Design review of the part built by this model. Coordinates are the model's own, in mm. A direction names the side the tool comes from. Give positions to 0.01 mm unless a question says otherwise; leave off trailing zeros. Loops run counter-clockwise (first coordinate to the right, second up) from the corner with the lowest first, then second, coordinate; pieces in that order, holes last.
from build123d import *

# Parameters (mm, degrees)
SKETCH_1_R      = 6
EXTRUDE_1_DEPTH = 120
SKETCH_2_R      = 4
EXTRUDE_2_DEPTH = 12
EXTRUDE_START   = 25
SKETCH_3_R      = 4
EXTRUDE_3_DEPTH = 25


with BuildPart() as part:
    # 草图1 → 凸台-拉伸1 (new body)
    with BuildSketch(Plane.XY):
        Circle(SKETCH_1_R)
    extrude(amount=EXTRUDE_1_DEPTH)

    # 草图2 → 凸台-拉伸2 (add)
    with BuildSketch(Plane(origin=(0, 0, 0), x_dir=(-1, 0, 0), z_dir=(0, 0, -1))):
        Circle(SKETCH_2_R)
    extrude(amount=EXTRUDE_2_DEPTH)

    # 草图3 → 凸台-拉伸3 (add)
    with BuildSketch(Plane.XY.offset(120).offset(EXTRUDE_START)):
        with Locations(Location((0, 0, 0), (0, 0, 180))):
            Circle(SKETCH_3_R)
    extrude(amount=-EXTRUDE_3_DEPTH)


solid = part.part
Q1. Tool access review of faces 1 (the face through (0.867, -3.905, -5.916)), 2 (the face through (0.867, 3.905, 132.675)), 3 (the face through (-6, 0, 59)): name each direction out of +Z, -Z, +X, -X, +Y, -Y from which nothing blocks a thin tool from reaching the whole face with its end or side.
Results:
face 1: -Z
face 2: +Z
face 3: +Z, -Z
Q2. Take a section at A-A (y = 0). Give the boundary of the cut face in (x, z).
Results:
outline: (-6, 0) - (-4, 0) - (-4, -12) - (4, -12) - (4, 0) - (6, 0) - (6, 120) - (4, 120) - (4, 145) - (-4, 145) - (-4, 120) - (-6, 120) - close
Q3. Wall thickness on line 1 (Z direction, x = 3.5, y = -2); line 2 (X direction, y = 4.5, z = 7); line 3 (X direction, y = 0.5, z = 39): over which ranges is each line inside the solid? List them lowest first.
Results:
line 1: z = 0 to 120
line 2: x = -3.97 to 3.97
line 3: x = -5.98 to 5.98
